The model under review builds one solid part; all positions refer to its coordinate system, in mm. A direction names the side the tool comes from. Coordinates: 2 decimals unless noted, no trailing zeros. Loops run counter-clockwise (first coordinate to the right, second up) from the corner with the lowest first, then second, coordinate; pieces in that order, holes last. Notation, with made-up numbers: (15.25, 75.5) - (26.25, 75.5) arc R32 cw to (26.25, 109.5) - close; hole circle Ø5 at (42, 2). An arc over 180 degrees is marked (long way). Answer in a Markdown table with one row per item. Add a question column.
(1) We need section B-B on z = 36. Write out the cut boundary in (x, y).
(2) We need section A-A on y = 0. Write out the cut boundary in (x, z), plus the area to 3 significant figures.
(3) Machinability: for faces 5 (the cylindrical face through (345.994, 0.572, 39.44)), 6 (the cylindrical face through (344.994, 0.55, 39.44)), which of the approach directions +Z, -Z, +X, -X, +Y, -Y give a long, thin tool a straight path to every point of the face, cutting with its end or side? Answer none if there is none.
(4) We need section C-C on x = 248. Write out the cut boundary in (y, z).
(5) For P1, Ø2, axis at y = -6, z = 15.5, coming from the +X side; P2, Ø3, axis at y = -20.5, z = 13.5, coming from the -X side, all flat-tipped, find the tip position at first contact; note any pin that passes through.
(6) For line 1 along Y through (x, z) = (60.5, 29.5); line 2 along X through (y, z) = (6, 25.5); line 3 along X through (y, z) = (17.5, 18), list the stretches that pass through material, from the lowest coordinate up.
(7) Mouldability with a two-part tool opening along Y and no side actions: class faces 1 (the flat face through (160.9, 25.2, 80)), 2 (the flat face through (158, 26, 39)), 3 (the cylindrical face through (-25.994, -0.572, 39.44)), 4 (the cylindrical face through (-24.994, -0.55, 39.44)) as +Y half, -Y half, draft (parallel to the pull), parting line (faces both ways), or undercut.
from build123d import *

# Parameters (mm, degrees)
BOSS_EXTRUDE1_DEPTH = 80


with BuildPart() as part:
    # Sketch1 → Boss-Extrude1 (new body)
    with BuildSketch(Plane.XY):
        with BuildLine():
            Line((320, -26), (0, -26))
            ThreePointArc((0, -26), (-26, 0), (0, 26))
            Line((0, 26), (320, 26))
            ThreePointArc((320, 26), (346, 0), (320, -26))
        make_face()
        with BuildLine():
            Line((0, 25), (320, 25))
            ThreePointArc((320, 25), (345, 0), (320, -25))
            Line((320, -25), (0, -25))
            ThreePointArc((0, -25), (-25, 0), (0, 25))
        make_face(mode=Mode.SUBTRACT)
    extrude(amount=BOSS_EXTRUDE1_DEPTH)


solid = part.part
Outcome:
| question | item | result |
|---|---|---|
| 1 | outline | (0, -26) - (320, -26) arc R26 ccw to (320, 26) - (0, 26) arc R26 ccw to start; hole (0, -25) - (320, -25) arc R25 ccw to (320, 25) - (0, 25) arc R25 ccw to start |
| 2 | outline | (-26, 0) - (-25, 0) - (-25, 80) - (-26, 80) - close; (345, 0) - (346, 0) - (346, 80) - (345, 80) - close |
| 2 | area | 160 mm² |
| 3 | face 5 | +Z, -Z, +X |
| 3 | face 6 | +Z, -Z |
| 4 | outline | (-26, 0) - (-25, 0) - (-25, 80) - (-26, 80) - close; (25, 0) - (26, 0) - (26, 80) - (25, 80) - close |
| 5 | P1 | x = 345.51 |
| 5 | P2 | x = -17.75 |
| 6 | line 1 | -26 to -25, 25 to 26 |
| 6 | line 2 | -25.3 to -24.27, 344.27 to 345.3 |
| 6 | line 3 | -19.23 to -17.85, 337.85 to 339.23 |
| 7 | face 1 | draft |
| 7 | face 2 | +Y half |
| 7 | face 3 | parting line |
| 7 | face 4 | undercut |
